Geometry check sheet. Reference: the model listing, model coordinates, mm. A direction names the side the tool comes from. Give positions to 0.01 mm unless a question says otherwise; leave off trailing zeros. Write each loop counter-clockwise with the first axis right and the second up, starting at its lowest first coordinate (ties: lowest second). Pieces come first, ordered by that corner, then holes. Notation, with made-up numbers: (87, -12.5) -> (141, -12.5) arc R20 cw to (141, -0.5) -> close; hole circle Ø2 at (61.25, 0.25). An arc over 180 degrees is marked (long way). Write item = value, one per line. Start each with the question number.
1. Set-up check for faces 4 (the flat face through (0, 730, 175)), 5 (the flat face through (0, 342.5, 86)): record each of +Z, -Z, +X, -X, +Y, -Y from which the full face is reachable in a straight line by a thin tool's end or side.
2. Depth check by flat-ended pin: P1, Ø4.5, axis at x = -2.5, y = 470.5, coming from the +Z side; P2, Ø7.5, axis at x = 1, y = 403.5, coming from the -Z side; P3, Ø4, axis at x = 2, z = 75, coming from the +Y side. Enter the tip coordinate at first touch or a pass-through.
3. Mould release check, pull along Z, two halves, no side actions. Record for faces 1 (the flat face through (0, 357.5, 86)), 2 (the flat face through (0, 370, 182.5)), 3 (the flat face through (0, 360, -7.5)): pulls with the +Z half, pulls with the -Z half, needs draft (parallel to the pull), parting line crosses it, or undercut.
4. Cross-section at A-A, the plane y = 60. Record the cut outline in (x, z), plus the area to 3 significant figures.
5. Thickness scan on line 1 along Z through (x, y) = (5, 286); line 2 along Y through (x, z) = (-1, 186); line 3 along Y through (x, z) = (0, 185). Record the ranges inside material, lowest first.
6. Cross-section at B-B, the plane z = -30. Record the cut outline in (x, y).
```python
from build123d import *

# Parameters (mm, degrees)
SKETCH1_W                = 15
SKETCH1_H                = 15
BOSS_EXTRUDE1_DEPTH      = 730
SKETCH2_R                = 5
BOSS_EXTRUDE2_DEPTH      = 8
SKETCH4_W                = 15
SKETCH4_H                = 15
BOSS_EXTRUDE3_DEPTH      = 160
SKETCH5_W                = 15
SKETCH5_H                = 730
BOSS_EXTRUDE4_DEPTH      = 15
BOSS_EXTRUDE5_START      = 8
SKETCH6_R                = 5
BOSS_EXTRUDE5_DEPTH      = 8
FILLET1_R                = 6
BOSS_EXTRUDE6_DEPTH      = 230
BOSS_EXTRUDE6_DEPTH_BACK = 55
SKETCH7_R                = 4


with BuildPart() as part:
    # Sketch1 → Boss-Extrude1 (new body)
    with BuildSketch(Plane(origin=(0, 0, 0), x_dir=(1, 0, 0), z_dir=(0, 1, 0))):
        Rectangle(SKETCH1_W, SKETCH1_H)
    extrude(amount=BOSS_EXTRUDE1_DEPTH)

    # Sketch2 → Boss-Extrude2 (add)
    with BuildSketch(Plane(origin=(0, 0, -7.5), x_dir=(-1, 0, 0), z_dir=(0, 0, -1))):
        with Locations(Location((0, 10, 0), (0, 0, 180))):
            Circle(SKETCH2_R)
    extrude(amount=BOSS_EXTRUDE2_DEPTH)

    # Sketch4 → Boss-Extrude3 (add)
    with BuildSketch(Plane.XY.offset(7.5)):
        with Locations((0, 350)):
            Rectangle(SKETCH4_W, SKETCH4_H)
    extrude(amount=BOSS_EXTRUDE3_DEPTH)

    # Sketch5 → Boss-Extrude4 (add)
    with BuildSketch(Plane.XY.offset(167.5)):
        with Locations((0, 365)):
            Rectangle(SKETCH5_W, SKETCH5_H)
    extrude(amount=BOSS_EXTRUDE4_DEPTH)

    # Sketch6 → Boss-Extrude5 (add)
    with BuildSketch(Plane.XY.offset(182.5).offset(BOSS_EXTRUDE5_START)):
        with Locations((0, 10)):
            Circle(SKETCH6_R)
    extrude(amount=-BOSS_EXTRUDE5_DEPTH)

    # Fillet1
    fillet1_edges = [part.edges().sort_by_distance(p)[0] for p in [
        (7.5, 0, 175),
        (-7.5, 0, 175),
        (-7.5, 0, 0),
        (7.5, 0, 0),
    ]]
    fillet(fillet1_edges, radius=FILLET1_R)

    # Sketch7 → Boss-Extrude6 (add, two sides: drawn at the far end of the back side and taken through both)
    with BuildSketch(Plane.XY.offset(7.5).offset(-BOSS_EXTRUDE6_DEPTH_BACK)):
        with Locations((0, 720)):
            Circle(SKETCH7_R)
    extrude(amount=BOSS_EXTRUDE6_DEPTH + BOSS_EXTRUDE6_DEPTH_BACK)


solid = part.part
```
Answers:
q1.face_4 = +Z, -Z, +X, -X, +Y
q1.face_5 = +X, -X, -Y
q2.P1 = 182.5
q2.P2 = -7.5
q2.P3 = 724
q3.face_1 = undercut
q3.face_2 = pulls with the +Z half
q3.face_3 = pulls with the -Z half
q4.outline = (-7.5, -7.5) -> (7.5, -7.5) -> (7.5, 7.5) -> (-7.5, 7.5) -> close; (-7.5, 167.5) -> (7.5, 167.5) -> (7.5, 182.5) -> (-7.5, 182.5) -> close
q4.area = 450 mm^2
q5.line_1 = -7.5 to 7.5, 167.5 to 182.5
q5.line_2 = 5.1 to 14.9, 716.13 to 723.87
q5.line_3 = 5 to 15, 716 to 724
q6.outline = circle Ø8 at (0, 720)
